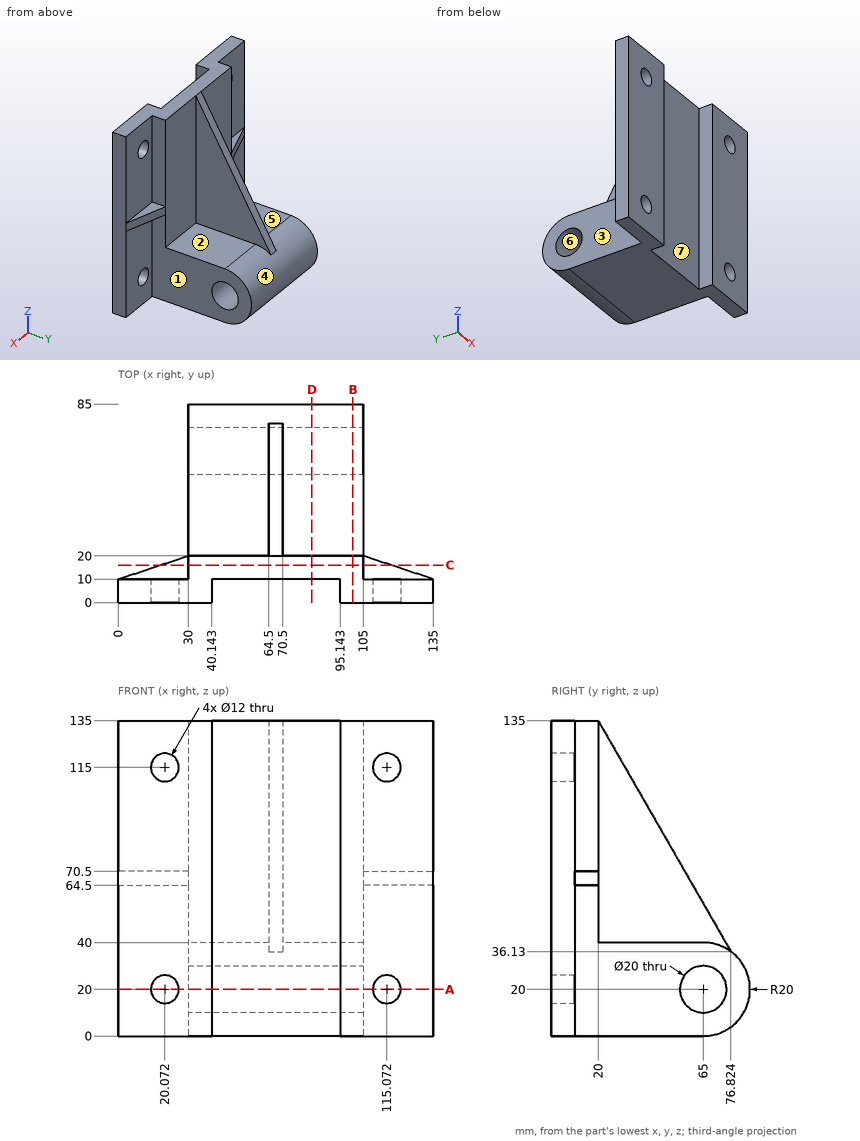
Geometry check sheet. Reference: drawing and pictorial views, mm from the part's lowest x, y, z. A direction names the side the tool comes from. Round coordinates to 2 decimals unless told otherwise and drop trailing zeros. Order: outer loops, then holes, each group sorted by start corner. A loop starts at its lowest first (then second) coordinate and runs counter-clockwise, first axis right, second up.
Q1. Cross-section at D-D, the plane x = 83. Enter the section's corners in (y, z).
Filled sheet:
outline: (10, 0) - (65, 0) arc R20 ccw to (65, 40) - (20, 40) - (20, 135) - (10, 135) - close; hole circle Ø20 at (65, 20)
Q2. Set-up check for the marked faces 1, 2 and 3: record each of +Z, -Z, +X, -X, +Y, -Y from which the full face is reachable in a straight line by a thin tool's end or side.
Filled sheet:
face 1: -Z, +X, +Y
face 2: +Z, +X, +Y
face 3: -Z, -X, +Y
Q3. Cross-section at C-C, the plane y = 16. Enter the section's corners in (x, z), plus the area to 3 significant figures.
Filled sheet:
outline: (18, 64.5) - (30, 64.5) - (30, 0) - (105, 0) - (105, 64.5) - (117, 64.5) - (117, 70.5) - (105, 70.5) - (105, 135) - (30, 135) - (30, 70.5) - (18, 70.5) - close
area: 10,300 mm2
Q4. Depth check by flat-ended pin: P1, Ø1.5, axis at y = 12, z = 62.5, coming from the +X side; P2, Ø6, axis at x = 40, y = 70, coming from the -Z side; P3, Ø11, axis at x = 123, y = 14, coming from the -Z side; P4, Ø16.5, axis at x = 61, z = 90.5, coming from the -Y side. Enter the tip coordinate at first touch or a pass-through.
Filled sheet:
P1: stops at x = 105
P2: stops at z = 0.1
P3: stops at z = 0
P4: stops at y = 10
Q5. Cross-section at B-B, the plane x = 100.5. Enter the section's corners in (y, z), plus the area to 3 significant figures.
Filled sheet:
outline: (0, 0) - (65, 0) arc R20 ccw to (65, 40) - (20, 40) - (20, 135) - (0, 135) - close; hole circle Ø20 at (65, 20)
area: 4,810 mm2
Q6. Draft check along Z on the marked faces 4, 5, 6 and 7. Enter one of: pulls with the +Z half, pulls with the -Z half, needs draft (parallel to the pull), parting line crosses it, or undercut.
Filled sheet:
face 4: parting line crosses it
face 5: pulls with the +Z half
face 6: undercut
face 7: needs draft
Q7. Cross-section at A-A, the plane z = 20. Enter the section's corners in (x, y).
Filled sheet:
outline: (0, 0) - (14.07, 0) - (14.07, 10) - (0, 10) - close; (26.07, 0) - (40.14, 0) - (40.14, 10) - (95.14, 10) - (95.14, 0) - (109.07, 0) - (109.07, 10) - (105, 10) - (105, 55) - (30, 55) - (30, 10) - (26.07, 10) - close; (30, 75) - (105, 75) - (105, 85) - (30, 85) - close; (121.07, 0) - (135, 0) - (135, 10) - (121.07, 10) - close
Q8. Scan lines: L1, parallel to X at y = 2, z = 115; L2, parallel to Y at x = 46, z = 20; L3, parallel to X at y = 9.5, z = 119 (1 decimal). Record each from-to range of solid material in increasing order.
Filled sheet:
L1: x = 0 to 14.07, 26.07 to 40.14, 95.14 to 109.07, 121.07 to 135
L2: y = 10 to 55, 75 to 85
L3: x = 0 to 15.6, 24.5 to 40.1, 95.1 to 110.6, 119.5 to 135
